CAD build for the part. Positions are in the model's coordinates, mm. A direction names the side the tool comes from. Give positions to 0.01 mm unless a question says otherwise; leave off trailing zeros. Write each loop counter-clockwise with the first axis right and the second up, starting at its lowest first coordinate (ties: lowest second). Pieces come first, ordered by that corner, then holes. Notation, with made-up numbers: (15, -37.75) - (42, -37.75) arc R20 cw to (42, -5.75) - close; hole circle Ø1 at (40.25, -23.75). An arc over 180 degrees is marked (long way). Answer as a JSON object with one key per item and string values.
from build123d import *

# Parameters (mm, degrees)
COLUMN_BASE_SKETCH_R    = 45
COLUMN_BASE_90_DEPTH    = 25
GROOVE_NECK_SKETCH_R    = 40
GROOVE_NECK_80_DEPTH    = 10
COLUMN_BODY_SKETCH_R    = 45
COLUMN_BODY_90_DEPTH    = 80
TOP_PLATE_170X130_DEPTH = 20
BORE_STEP_SKETCH_R      = 28
BORE_STEP_28_DEPTH      = 15
COLUMN_BORE_SKETCH_R    = 20
COLUMN_BORE_40_DEPTH    = 150
PLATE_HOLES_SKETCH_R    = 15
PLATE_HOLES_SKETCH_R_2  = 10
PLATE_HOLES_6X_DEPTH    = 150
EYE_LUG_DEPTH           = 15
LUG_HOLE_SKETCH_R       = 10
LUG_HOLE_10_DEPTH       = 15


with BuildPart() as part:
    # Column Base Sketch → Column Base Ø90 (new body)
    with BuildSketch(Plane.XY):
        Circle(COLUMN_BASE_SKETCH_R)
    extrude(amount=COLUMN_BASE_90_DEPTH)

    # Groove Neck Sketch → Groove Neck Ø80 (add)
    with BuildSketch(Plane.XY.offset(25)):
        Circle(GROOVE_NECK_SKETCH_R)
    extrude(amount=GROOVE_NECK_80_DEPTH)

    # Column Body Sketch → Column Body Ø90 (add)
    with BuildSketch(Plane.XY.offset(35)):
        Circle(COLUMN_BODY_SKETCH_R)
    extrude(amount=COLUMN_BODY_90_DEPTH)

    # Top Plate Sketch → Top Plate 170x130 (add)
    with BuildSketch(Plane.XY.offset(115)):
        with BuildLine():
            Line((70, 65), (0, 65))
            Line((0, 65), (-70, 65))
            ThreePointArc((-70, 65), (-80.606601718, 60.606601718), (-85, 50))
            Line((-85, 50), (-85, -50))
            ThreePointArc((-85, -50), (-80.606601718, -60.606601718), (-70, -65))
            Line((-70, -65), (70, -65))
            ThreePointArc((70, -65), (80.606601718, -60.606601718), (85, -50))
            Line((85, -50), (85, 50))
            ThreePointArc((85, 50), (80.606601718, 60.606601718), (70, 65))
        make_face()
    extrude(amount=TOP_PLATE_170X130_DEPTH)

    # Bore Step Sketch → Bore Step Ø28 (cut)
    with BuildSketch(Plane.XY.offset(135)):
        Circle(BORE_STEP_SKETCH_R)
    extrude(amount=-BORE_STEP_28_DEPTH, mode=Mode.SUBTRACT)

    # Column Bore Sketch → Column Bore Ø40 (cut)
    with BuildSketch(Plane.XY.offset(120)):
        Circle(COLUMN_BORE_SKETCH_R)
    extrude(amount=-COLUMN_BORE_40_DEPTH, mode=Mode.SUBTRACT)

    # Plate Holes Sketch → Plate Holes 6x (cut)
    with BuildSketch(Plane.XY.offset(135)):
        with Locations((-55, 35)):
            Circle(PLATE_HOLES_SKETCH_R)
        with Locations((55, 35)):
            Circle(PLATE_HOLES_SKETCH_R)
        with Locations((-55, -35)):
            Circle(PLATE_HOLES_SKETCH_R)
        with Locations((55, -35)):
            Circle(PLATE_HOLES_SKETCH_R)
        with Locations((-55, 0)):
            Circle(PLATE_HOLES_SKETCH_R_2)
        with Locations((55, 0)):
            Circle(PLATE_HOLES_SKETCH_R_2)
    extrude(amount=-PLATE_HOLES_6X_DEPTH, mode=Mode.SUBTRACT)

    # Eye Lug Sketch → Eye Lug (add)
    with BuildSketch(Plane.XZ.offset(65)):
        with BuildLine():
            Line((-15, 135), (15, 135))
            Line((15, 135), (15, 155))
            ThreePointArc((15, 155), (0, 170), (-15, 155))
            Line((-15, 155), (-15, 135))
        make_face()
    extrude(amount=-EYE_LUG_DEPTH)

    # Lug Hole Sketch → Lug Hole Ø10 (cut)
    with BuildSketch(Plane(origin=(0, -50, 0), x_dir=(1, 0, 0), z_dir=(0, 1, 0))):
        with Locations(Location((0, -155, 0), (0, 0, 270))):
            Circle(LUG_HOLE_SKETCH_R)
    extrude(amount=-LUG_HOLE_10_DEPTH, mode=Mode.SUBTRACT)


solid = part.part
(1) Saw through at B-B, the plane y = -35. Give the cut face in (x, z), and give its area (3 significant figures).
Answer key:
{"outline": "(-85, 115) - (-70, 115) - (-70, 135) - (-85, 135) - close; (-40, 115) - (-28.28, 115) - (-28.28, 35) - (-19.36, 35) - (-19.36, 25) - (-28.28, 25) - (-28.28, 0) - (28.28, 0) - (28.28, 25) - (19.36, 25) - (19.36, 35) - (28.28, 35) - (28.28, 115) - (40, 115) - (40, 135) - (-40, 135) - close; (70, 115) - (85, 115) - (85, 135) - (70, 135) - close", "area": "8,530 mm²"}
(2) Saw through at C-C, the plane x = -55. Give the cut face in (y, z).
Answer key:
{"outline": "(-65, 115) - (-50, 115) - (-50, 135) - (-65, 135) - close; (-20, 115) - (-10, 115) - (-10, 135) - (-20, 135) - close; (10, 115) - (20, 115) - (20, 135) - (10, 135) - close; (50, 115) - (65, 115) - (65, 135) - (50, 135) - close"}
(3) 3-axis set-ups, long thin cutter, end or side, ignore diameter. For faces 1 (the face through (-15, -58, 145)), 2 (the face through (-30.2, -26.5, 25)), 3 (the face through (20.765, -39.923, 12.325)): which of +Z, -Z, +X, -X, +Y, -Y reach the whole face in a straight line?
Answer key:
{"face 1": "+Z, -X, +Y, -Y", "face 2": "none", "face 3": "-Z"}
(4) Pull direction Y, two halves, no side cores. Call faces 4 (the face through (-66.056, -24.862, 125.14)), 5 (the face through (-20, 44, 115)), 6 (the face through (80.72, 60.49, 124.86)): pulls with the +Y half, pulls with the -Y half, needs draft (parallel to the pull), parting line crosses it, or undercut.
Answer key:
{"face 4": "undercut", "face 5": "needs draft", "face 6": "pulls with the +Y half"}
(5) Saw through at D-D, the plane z = 104. Give the cut face in (x, y).
Answer key:
{"outline": "circle Ø90 at (0, 0); hole circle Ø40 at (0, 0)"}
(6) Probe L1, parallel to Y at x = 55, z = 121.25; L2, parallel to Y at x = 0, z = 127; L3, parallel to X at y = -59.25, z = 155. List the from-to ranges inside material, lowest first. Write a range as [from, to].
Answer key:
{"L1": "y = [-65, -50], [-20, -10], [10, 20], [50, 65]", "L2": "y = [-65, -28], [28, 65]", "L3": "x = [-15, -10], [10, 15]"}
(7) Saw through at A-A, the plane x = 0. State how many separate pieces and enclosed holes the cut face has, and give its area (4 significant figures).
Answer key:
{"separate pieces": "3", "enclosed holes": "0", "area": "7,435 mm²"}
(8) Flat gauge pins, fed straight in: P1, Ø3, axis at x = -12.5, z = 148, coming from the +Y side; P2, Ø18, axis at x = -55, y = 35, coming from the -Z side; P3, Ø23, axis at x = -55, y = 0, coming from the +Z side; P4, Ø5, axis at x = 42, z = 41, coming from the +Y side. Where does each tip first touch, or does it go through?
Answer key:
{"P1": "stops at y = -50", "P2": "passes through", "P3": "stops at z = 135", "P4": "stops at y = 21.56"}
